from build123d import *

# Parameters (mm, degrees)
SKETCH_3_R          = 10
EXTRUDE_3_DEPTH     = 185
CUT_EXTRUDE_1_DEPTH = 12.5
SKETCH_5_W          = 370
SKETCH_5_H          = 20
CUT_EXTRUDE_2_DEPTH = 10


with BuildPart() as part:
    # 草图3 → 凸台-拉伸3 (new, symmetric)
    with BuildSketch(Plane.XY):
        Circle(SKETCH_3_R)
    extrude(amount=EXTRUDE_3_DEPTH, both=True)

    # 草图4 → 切除-拉伸1 (cut, symmetric)
    with BuildSketch(Plane(origin=(0, 0, 0), x_dir=(1, 0, 0), z_dir=(0, 1, 0))):
        with BuildLine():
            Line((-2, -160), (-2, 160))
            ThreePointArc((-2, 160), (0, 162), (2, 160))
            Line((2, 160), (2, -160))
            ThreePointArc((2, -160), (0, -162), (-2, -160))
        make_face()
    extrude(amount=CUT_EXTRUDE_1_DEPTH, both=True, mode=Mode.SUBTRACT)

    # 草图5 → 切除-拉伸2 (cut, symmetric)
    with BuildSketch(Plane(origin=(0, 0, 0), x_dir=(0, 0, -1), z_dir=(1, 0, 0))):
        with Locations((0, 14)):
            Rectangle(SKETCH_5_W, SKETCH_5_H)
    extrude(amount=CUT_EXTRUDE_2_DEPTH, both=True, mode=Mode.SUBTRACT)


solid = part.part
Source: CAD feature listing. Evaluate the final solid. Frame: model axes, mm. Coordinates: 2 decimals unless noted, no trailing zeros. Loops run counter-clockwise (first coordinate to the right, second up) from the corner with the lowest first, then second, coordinate; pieces in that order, holes last. Notation, with made-up numbers: (4.5, -4) - (49.5, -4) arc R28 ccw to (49.5, 17) - close; hole circle Ø1 at (25, 46.25). An arc over 180 degrees is marked (long way). One line per question, with ' | ' between items.
1) Line query: line 1 along X through (y, z) = (-1, -154.5); line 2 along Z through (x, y) = (-0.5, 3.25); line 3 along X through (y, z) = (0.75, 123.5). Output: solid intervals per line, ascending.
Report:
line 1: x = -9.95 to -2, 2 to 9.95 | line 2: z = -185 to -161.94, 161.94 to 185 | line 3: x = -9.97 to -2, 2 to 9.97
2) Section B-B, the plane z = -137.5. Return loops of the section in (x, y), then the cut area to 3 significant figures.
Report:
outline: (-9.17, 4) arc R10 ccw to (-2, -9.8) - (-2, 4) - close; (2, -9.8) arc R10 ccw to (9.17, 4) - (2, 4) - close | area: 179 mm²
3) Pull-direction query (Z, two-part tool) for faces 1 (the face through (-2, -3, 2)), 2 (the face through (2, -3, -2)), 3 (the face through (0, -1, -185)), 4 (the face through (0, -1, 185)); classes: released by +Z, released by -Z, zero draft, split by the parting line, or undercut.
Report:
face 1: undercut | face 2: undercut | face 3: released by -Z | face 4: released by +Z
4) Section A-A, the plane y = 0. Return loops of the section in (x, z).
Report:
outline: (-10, -185) - (10, -185) - (10, 185) - (-10, 185) - close; hole (-2, -160) arc R2 ccw to (2, -160) - (2, 160) arc R2 ccw to (-2, 160) - close
5) First-contact query: P1, Ø10, axis at x = -3, z = -110, coming from the -Y side. Flat tip, straight axial feed; report the tip coordinate or a pass-through.
Report:
P1: stops at y = -9.8
